from build123d import *

# Parameters (mm, degrees)
BASE_PLATE_DEPTH          = 26
U_POCKET_14_DEEP_DEPTH    = 14
ANGLED_TAB_30DEG_DEPTH    = 12
BOSS_CIRCLE_SKETCH_R      = 17
BOSS_34_DEPTH             = 30
BOSS_BORE_SKETCH_R        = 6
BOSS_BORE_12_DEPTH        = 141.220821249
TAB_HOLES_SKETCH_R        = 14
TAB_HOLES_SKETCH_R_2      = 6
TAB_HOLES_28_AND_12_DEPTH = 30


with BuildPart() as part:
    # Base Profile Sketch → Base Plate (new body)
    with BuildSketch(Plane(origin=(0, 0, 0), x_dir=(1, 0, 0), z_dir=(0, 1, 0))):
        with BuildLine():
            Line((0, 34), (59.4, 34))
            Line((59.4, 34), (59.4, -34))
            Line((59.4, -34), (0, -34))
            ThreePointArc((0, -34), (-34, 0), (0, 34))
        make_face()
    extrude(amount=BASE_PLATE_DEPTH)

    # Pocket Profile Sketch → U Pocket 14 Deep (cut)
    with BuildSketch(Plane(origin=(0, 26, 0), x_dir=(1, 0, 0), z_dir=(0, 1, 0))):
        with BuildLine():
            Line((0, 24), (59.4, 24))
            Line((59.4, 24), (59.4, -24))
            Line((59.4, -24), (0, -24))
            ThreePointArc((0, -24), (-24, 0), (0, 24))
        make_face()
    extrude(amount=-U_POCKET_14_DEEP_DEPTH, mode=Mode.SUBTRACT)

    # Angled Tab Sketch → Angled Tab 30deg (add)
    with BuildSketch(Plane(origin=(0, 12, 0), x_dir=(1, 0, 0), z_dir=(0, 1, 0))):
        Polygon((59.4, 34), (122.619854476, -2.5), (93.174990748, -53.5), (59.4, -34), align=None)
    extrude(amount=-ANGLED_TAB_30DEG_DEPTH)

    # Boss Circle Sketch → Boss Ø34 (add)
    with BuildSketch(Plane(origin=(0, 12, 0), x_dir=(1, 0, 0), z_dir=(0, 1, 0))):
        with Locations(Location((0, 0, 0), (0, 0, 270))):
            Circle(BOSS_CIRCLE_SKETCH_R)
    extrude(amount=BOSS_34_DEPTH)

    # Boss Bore Sketch → Boss Bore Ø12 (cut, through all)
    with BuildSketch(Plane(origin=(0, 42, 0), x_dir=(1, 0, 0), z_dir=(0, 1, 0))):
        with Locations(Location((0, 0, 0), (0, 0, 270))):
            Circle(BOSS_BORE_SKETCH_R)
    extrude(amount=-BOSS_BORE_12_DEPTH, mode=Mode.SUBTRACT)

    # Tab Holes Sketch → Tab Holes Ø28 and Ø12 (cut)
    with BuildSketch(Plane(origin=(0, 12, 0), x_dir=(1, 0, 0), z_dir=(0, 1, 0))):
        with Locations(Location((59.4, 0, 0), (0, 0, 270))):
            Circle(TAB_HOLES_SKETCH_R)
        with Locations(Location((90.576914536, -18, 0), (0, 0, 270))):
            Circle(TAB_HOLES_SKETCH_R_2)
    extrude(amount=-TAB_HOLES_28_AND_12_DEPTH, mode=Mode.SUBTRACT)


solid = part.part
Work out the finished part from the listing and answer in its coordinate system (mm). A direction names the side the tool comes from. Round coordinates to 2 decimals unless told otherwise and drop trailing zeros. Loops run counter-clockwise (first coordinate to the right, second up) from the corner with the lowest first, then second, coordinate; pieces in that order, holes last. Notation, with made-up numbers: M 71.25,89.5 L 95.25,89.5 A16 ccw 95.25,98.5 Z; hole C 15.25,11.25 d1. An arc over 180 degrees is marked long. One line per question, with ' | ' between items. Start each with the question number.
(1) A cutting plane is placed at C-C on z = 0. Write down the section's boundary in (x, y).
(2) A tool of negligible diameter and unlimited length cuts with its end or side. For faces 1 (the face through (30, 19, 24)), 2 (the face through (-23.994, 19.098, 0.528)), 3 (the face through (59.4, 19, 29)), from which of +Z, -Z, +X, -X, +Y, -Y can it reach the whole face along a straight path? Write none if from no direction.
(3) Flat-ended cylindrical pins translate along their axes: pin 1 Ø5 at (y, z) = (26.5, 12.5) entering from +X; pin 2 Ø7 at (x, y) = (16.5, 20.5) entering from +Z; pin 3 Ø4 at (x, y) = (-4, 32) entering from +Z. Find the tip coordinate at first contact, or state that the pin passes through.
(4) A cutting plane is placed at B-B on x = 54.5. Write down the section's boundary in (y, z), plus the area to 3 significant figures.
(5) A cutting plane is placed at D-D on y = 29. Write down the section's boundary in (x, z), plus the area to 3 significant figures.
(6) Find the intervals of material crossed by line 1 (X direction, y = 22.5, z = 0); line 2 (X direction, y = 2, z = 1.5); line 3 (Z direction, x = 22, y = 21), in increasing order.
(7) A cutting plane is placed at A-A on y = 17. Write down the section's boundary in (x, z).
Geometry check:
1) outline: M -34,0 L -6,0 L -6,42 L -17,42 L -17,12 L -24,12 L -24,26 L -34,26 Z; M 6,0 L 45.4,0 L 45.4,12 L 17,12 L 17,42 L 6,42 Z; M 73.4,0 L 118.29,0 L 118.29,12 L 73.4,12 Z
2) face 1: +X, +Y | face 2: +Y | face 3: +Z, -Z, +X, +Y
3) pin 1: stops at x = 13.75 | pin 2: stops at z = 34 | pin 3: stops at z = 16.88
4) outline: M 0,-34 L 26,-34 L 26,-24 L 12,-24 L 12,-13.11 L 0,-13.11 Z; M 0,13.11 L 12,13.11 L 12,24 L 26,24 L 26,34 L 0,34 Z | area: 781 mm²
5) outline: C 0,0 d34; hole C 0,0 d12 | area: 795 mm²
6) line 1: x = -34 to -24, -17 to -6, 6 to 17 | line 2: x = -33.97 to -5.81, 5.81 to 45.48, 73.32 to 120.89 | line 3: z = -34 to -24, 24 to 34
7) outline: C 0,0 d34; M 0,-34 L 59.4,-34 L 59.4,-24 L 0,-24 A24 cw 0,24 L 59.4,24 L 59.4,34 L 0,34 A34 ccw Z; hole C 0,0 d12
